from build123d import *

# Parameters (mm, degrees)
SWEEP1_PROFILE_R    = 1
BOSS_EXTRUDE1_DEPTH = 1.5
BOSS_EXTRUDE2_DEPTH = 1


with BuildPart() as part:
    # Sketch1 → Revolve1 (revolve)
    with BuildSketch(Plane.XY, mode=Mode.PRIVATE) as revolve1_sk:
        Polygon((0, 0), (0, 2.5), (2, 2.5), (2, 5), (3, 5), (3, 0), align=None)
    revolve(revolve1_sk.sketch.rotate(Axis((0, 0, 0), (1, 0, 0)), 90), axis=Axis((0, 0, 0), (1, 0, 0)))

    # Sweep1: sweep along a path in Sketch2
    with BuildLine(Plane.XY) as sweep1_path:
        Line((3, 0), (53, 0))
        ThreePointArc((53, 0), (69.90473047, -3.747688519), (83.641777725, -14.288495613))
        Line((83.641777725, -14.288495613), (160.776290887, -106.213828787))
    # Sweep1 profile (on start of the path) → Sweep1 (sweep)
    with BuildSketch(Plane(origin=(3, 0, 0), x_dir=(0, 0, 1), z_dir=(1, 0, 0))):
        Circle(SWEEP1_PROFILE_R)
    sweep(path=sweep1_path.line)

    # Sketch11 → Boss-Extrude1 (add, symmetric)
    with BuildSketch(Plane.XY):
        Polygon((160.010246444, -106.856616397), (161.54233533, -105.571041177), (162.951167383, -105.694298011), (164.236742602, -107.226386897), (161.17256483, -109.797537336), (159.886989611, -108.265448449), align=None)
    extrude(amount=BOSS_EXTRUDE1_DEPTH, both=True)

    # Sketch12 → Boss-Extrude2 (add, symmetric)
    with BuildSketch(Plane.XY):
        Polygon((163.509000381, -107.837035126), (164.794575601, -109.369124012), (164.564762268, -109.561960295), (163.279187049, -108.029871409), align=None)
        Polygon((162.130120384, -108.994052823), (161.900307051, -109.186889106), (163.18588227, -110.718977993), (163.415695603, -110.52614171), align=None)
    extrude(amount=BOSS_EXTRUDE2_DEPTH, both=True)


solid = part.part
Source: CAD feature listing. Evaluate the final solid. Frame: model axes, mm. A direction names the side the tool comes from. Coordinates: 2 decimals unless noted, no trailing zeros. Loops run counter-clockwise (first coordinate to the right, second up) from the corner with the lowest first, then second, coordinate; pieces in that order, holes last. Notation, with made-up numbers: (6.5, 18) - (27.5, 18) arc R13 cw to (27.5, 41) - close; hole circle Ø1 at (-27, 49.25). An arc over 180 degrees is marked (long way). One line per item, written item: value. Start each with the question number.
1. Set-up query: faces 1 (the cylindrical face through (1, -0.1, -2.5)), 2 (the cylindrical face through (121.99, -61.53, -0.13)). Return all of +Z, -Z, +X, -X, +Y, -Y with unobstructed straight access to the full face (end or side cutting, diameter ignored); none if empty.
2. Contact query for flat-ended pins moving along their axis: P1, Ø1.2, axis at x = 164, y = -108.5, coming from the -Z side; P2, Ø2, axis at x = 162, y = -108, coming from the -Z side; P3, Ø0.8, axis at x = 163, y = -109.5, coming from the +Z side. Output: stop coordinate, or through.
3. Ray query, L1, parallel to X at y = -100, z = 0; L2, parallel to Y at x = 82, z = -0.5; L3, parallel to Y at x = 62.5, z = 0. Return the intervals inside material, ascending.
4. Section A-A (x = 10.5). Return the cut outline in (y, z).
Verdict:
1. face 1: -X
1. face 2: none
2. P1: stops at z = -1
2. P2: stops at z = -1.5
2. P3: stops at z = 1
3. L1: x = 154.26 to 156.87
3. L2: y = -13.72 to -11.21
3. L3: y = -2.17 to -0.12
4. outline: circle Ø2 at (0, 0)
